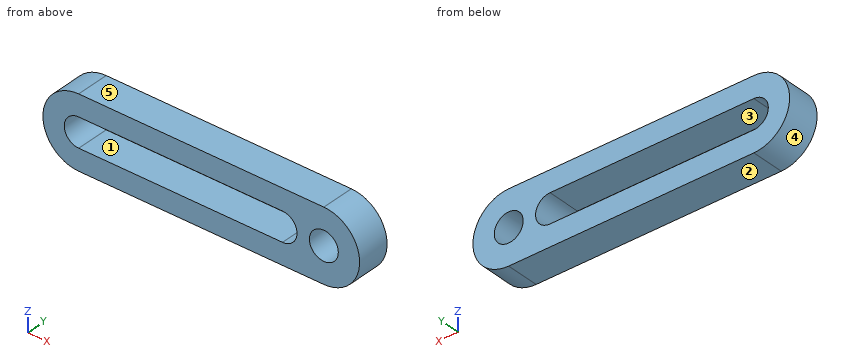
```python
from build123d import *

# Parameters (mm, degrees)
SKETCH1_R           = 5.25
BOSS_EXTRUDE1_DEPTH = 6


with BuildPart() as part:
    # Sketch1 → Boss-Extrude1 (new, symmetric)
    with BuildSketch(Plane(origin=(0, 0, 0), x_dir=(1, 0, 0), z_dir=(0, 1, 0))):
        with BuildLine():
            Line((-44.5, 13), (44.5, 13))
            ThreePointArc((44.5, 13), (57.5, 0), (44.5, -13))
            Line((44.5, -13), (-44.5, -13))
            ThreePointArc((-44.5, -13), (-57.5, 0), (-44.5, 13))
        make_face()
        with Locations(Location((44.5, 0, 0), (0, 0, 270))):
            Circle(SKETCH1_R, mode=Mode.SUBTRACT)
        with BuildLine():
            Line((-44.5, 5.25), (29.5, 5.25))
            ThreePointArc((29.5, 5.25), (34.75, 0), (29.5, -5.25))
            Line((29.5, -5.25), (-44.5, -5.25))
            ThreePointArc((-44.5, -5.25), (-49.75, 0), (-44.5, 5.25))
        make_face(mode=Mode.SUBTRACT)
    extrude(amount=BOSS_EXTRUDE1_DEPTH, both=True)


solid = part.part
```
Source: CAD feature listing. Evaluate the final solid. Frame: model axes, mm. Face numbers are marked on the shaded views. A direction names the side the tool comes from. Coordinates: 2 decimals unless noted, no trailing zeros. Loops run counter-clockwise (first coordinate to the right, second up) from the corner with the lowest first, then second, coordinate; pieces in that order, holes last. Notation, with made-up numbers: (84.25, 7) -> (107.25, 7) arc R15 cw to (107.25, 13) -> close; hole circle Ø2 at (-15.5, 72). An arc over 180 degrees is marked (long way). One line per item, written item: value. Start each with the question number.
Q1. Set-up query: the marked faces 1 and 2. Return all of +Z, -Z, +X, -X, +Y, -Y with unobstructed straight access to the full face (end or side cutting, diameter ignored); none if empty.
Q2. Section query B-B, the plane z = -2.25. Return the cut outline in (x, y).
Q3. Section query D-D, the plane z = 2.5. Return the cut outline in (x, y), and give its area (3 significant figures).
Q4. Section query C-C, the plane y = 4. Return the cut outline in (x, z).
Q5. Line query: line 1 along X through (y, z) = (-0.75, 0); line 2 along X through (y, z) = (3.5, -1.5); line 3 along Z through (x, y) = (-32, 5). Output: solid intervals per line, ascending.
Q6. Mould query, pull axis Z, two halves, no side actions, for the marked faces 3, 4 and 5. Classes: pulls with the +Z half, pulls with the -Z half, needs draft (parallel to the pull), parting line crosses it, or undercut.
Q7. Contact query for flat-ended pins moving along their axis: P1, Ø6, axis at y = -3, z = -7.5, coming from the -X side; P2, Ø4, axis at y = 3, z = -4.5, coming from the +X side; P3, Ø6, axis at y = -4, z = -3.5, coming from the +X side. Output: stop coordinate, or through.
Q8. Section query A-A, the plane x = -37.5. Return the cut outline in (y, z), and give its area (3 significant figures).
Results:
1. face 1: +Y, -Y
1. face 2: -Z, +X, -X, +Y, -Y
2. outline: (-57.3, -6) -> (-49.24, -6) -> (-49.24, 6) -> (-57.3, 6) -> close; (34.24, -6) -> (39.76, -6) -> (39.76, 6) -> (34.24, 6) -> close; (49.24, -6) -> (57.3, -6) -> (57.3, 6) -> (49.24, 6) -> close
3. outline: (-57.26, -6) -> (-49.12, -6) -> (-49.12, 6) -> (-57.26, 6) -> close; (34.12, -6) -> (39.88, -6) -> (39.88, 6) -> (34.12, 6) -> close; (49.12, -6) -> (57.26, -6) -> (57.26, 6) -> (49.12, 6) -> close
3. area: 265 mm^2
4. outline: (-44.5, -13) -> (44.5, -13) arc R13 ccw to (44.5, 13) -> (-44.5, 13) arc R13 ccw to start; hole (-44.5, -5.25) -> (29.5, -5.25) arc R5.25 ccw to (29.5, 5.25) -> (-44.5, 5.25) arc R5.25 ccw to start; hole circle Ø10.5 at (44.5, 0)
5. line 1: -57.5 to -49.75, 34.75 to 39.25, 49.75 to 57.5
5. line 2: -57.41 to -49.53, 34.53 to 39.47, 49.53 to 57.41
5. line 3: -13 to -5.25, 5.25 to 13
6. face 3: undercut
6. face 4: parting line crosses it
6. face 5: pulls with the +Z half
7. P1: x = -56.7
7. P2: x = 57.26
7. P3: x = 57.49
8. outline: (-6, -13) -> (6, -13) -> (6, -5.25) -> (-6, -5.25) -> close; (-6, 5.25) -> (6, 5.25) -> (6, 13) -> (-6, 13) -> close
8. area: 186 mm^2
